The model under review builds one solid part; all positions refer to its coordinate system, in mm. A direction names the side the tool comes from. Round coordinates to 2 decimals unless told otherwise and drop trailing zeros. Write each loop counter-clockwise with the first axis right and the second up, starting at its lowest first coordinate (ties: lowest second). Pieces come first, ordered by that corner, then holes. Notation, with made-up numbers: (55.5, -29) - (66.5, -29) arc R15 ccw to (66.5, -5) - close; hole circle Ø6 at (5.25, -20.5). An arc over 180 degrees is marked (long way). Use one line per item in the form item = value.
from build123d import *

# Parameters (mm, degrees)
SKETCH_2_R          = 1.5
CUT_EXTRUDE_1_DEPTH = 10


with BuildPart() as part:
    # 草图1 → 旋转1 (revolve)
    with BuildSketch(Plane.XY, mode=Mode.PRIVATE) as revolve_1_sk:
        Polygon((4, 7.261363636), (5.5, 7.261363636), (5.5, -0.738636364), (7, -0.738636364), (7, -5.238636364), (4, -5.238636364), align=None)
    revolve(revolve_1_sk.sketch.rotate(Axis((0, 0, 0), (0, 1, 0)), 90), axis=Axis((0, 0, 0), (0, 1, 0)))

    # 草图2 → 切除-拉伸1 (cut)
    with BuildSketch(Plane.XY):
        with Locations(Location((0, -2.988636364, 0), (0, 0, 270.000000001))):
            Circle(SKETCH_2_R)
    extrude(amount=-CUT_EXTRUDE_1_DEPTH, mode=Mode.SUBTRACT)


solid = part.part
(1) Machinability: for faces 5 (the flat face through (4, -0.739, -4)), 6 (the cylindrical face through (2.4, 1.1, 3.2)), which of the approach directions +Z, -Z, +X, -X, +Y, -Y give a long, thin tool a straight path to every point of the face, cutting with its end or side? Answer none if there is none.
Geometry results:
face_5 = +Y
face_6 = +Y, -Y
(2) To check wall thickness, follow L1, parallel to X at y = 3.25, z = 0; L2, parallel to X at y = -2.5, z = 0; L3, parallel to Y at x = -4.5, z = -5. State the ranges of each line that lie inside material, in increasing order.
Geometry results:
L1 = -5.5 to -4, 4 to 5.5
L2 = -7 to -4, 4 to 7
L3 = -5.24 to -0.74
(3) The part is to be moulded in two halves that separate along Y. For faces 1 (the flat face through (2, 7.261, -4)), 2 (the flat face through (3, -5.239, -3)), 3 (the cylindrical face through (-0.575, -4.374, -5.331)), 4 (the cylindrical face through (5.37, 3.21, 1.19)), say which applies: +Y half, -Y half, draft (parallel to the pull), parting line (faces both ways), or undercut.
Geometry results:
face_1 = +Y half
face_2 = -Y half
face_3 = undercut
face_4 = draft
(4) Add section D-D on x = -3.25. Write out the cut boundary in (y, z).
Geometry results:
outline = (-5.24, -6.2) - (-0.74, -6.2) - (-0.74, -4.44) - (7.26, -4.44) - (7.26, -2.33) - (-5.24, -2.33) - close; (-5.24, 2.33) - (7.26, 2.33) - (7.26, 4.44) - (-0.74, 4.44) - (-0.74, 6.2) - (-5.24, 6.2) - close
(5) Add section C-C on y = 1.5. Write out the cut boundary in (x, z).
Geometry results:
outline = circle Ø11 at (0, 0); hole circle Ø8 at (0, 0)
(6) Insertion check: P1, Ø1.5, axis at y = 3, z = 0, coming from the -X side; P2, Ø4, axis at x = -5, y = 4.5, coming from the +Z side. Each pin has a flat end and moves straight along its axis. Give the tip position at first contact, or say it passes through.
Geometry results:
P1 = -5.5
P2 = 4.61
(7) Add section B-B on x = 0. Write out the cut boundary in (y, z).
Geometry results:
outline = (-5.24, -7) - (-4.49, -7) - (-4.49, -4) - (-5.24, -4) - close; (-5.24, 4) - (7.26, 4) - (7.26, 5.5) - (-0.74, 5.5) - (-0.74, 7) - (-5.24, 7) - close; (-1.49, -7) - (-0.74, -7) - (-0.74, -5.5) - (7.26, -5.5) - (7.26, -4) - (-1.49, -4) - close
(8) Add section A-A on z = 0. Write out the cut boundary in (x, y).
Geometry results:
outline = (-7, -5.24) - (-4, -5.24) - (-4, 7.26) - (-5.5, 7.26) - (-5.5, -0.74) - (-7, -0.74) - close; (4, -5.24) - (7, -5.24) - (7, -0.74) - (5.5, -0.74) - (5.5, 7.26) - (4, 7.26) - close
